Part model, mm, in its own coordinate system. Face numbers are marked on the shaded views. Round coordinates to 2 decimals unless told otherwise and drop trailing zeros. Loops run counter-clockwise (first coordinate to the right, second up) from the corner with the lowest first, then second, coordinate; pieces in that order, holes last.
from build123d import *

# Parameters (mm, degrees)
SKETCH1_W           = 176
SKETCH1_H           = 176
BOSS_EXTRUDE1_DEPTH = 30
SKETCH3_R           = 5.055
CUT_EXTRUDE1_DEPTH  = 200.047732969


with BuildPart() as part:
    # Sketch1 → Boss-Extrude1 (new body)
    with BuildSketch(Plane.XY):
        Rectangle(SKETCH1_W, SKETCH1_H)
    extrude(amount=BOSS_EXTRUDE1_DEPTH)

    # Sketch3 → Cut-Extrude1 (cut, through all)
    with BuildSketch(Plane(origin=(0, 88, 0), x_dir=(1, 0, 0), z_dir=(0, 1, 0))):
        with Locations(Location((0, -15, 0), (0, 0, 180))):
            Circle(SKETCH3_R)
    extrude(amount=-CUT_EXTRUDE1_DEPTH, mode=Mode.SUBTRACT)


solid = part.part
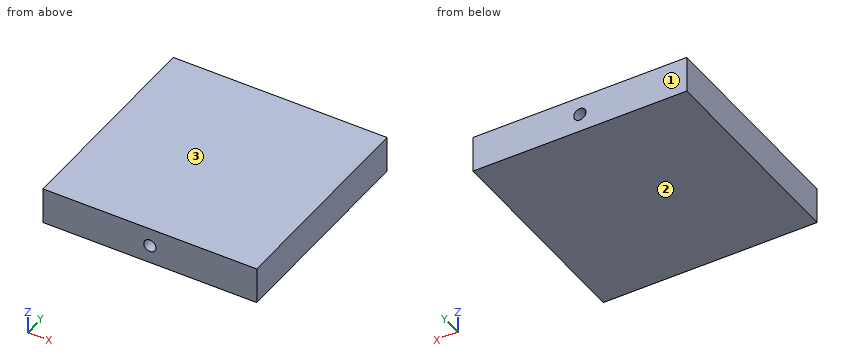
1) Mould opens along Z. For the marked faces 1, 2 and 3 say: released by +Z, released by -Z, zero draft, split by the parting line, or undercut.
Values:
face 1: zero draft
face 2: released by -Z
face 3: released by +Z
2) Slice it at B-B, the plane z = 15. Give the cut face in (x, y) (3 decimals), then the cut area to 3 significant figures.
Values:
outline: (-88, -88) - (-5.055, -88) - (-5.055, 88) - (-88, 88) - close; (5.055, -88) - (88, -88) - (88, 88) - (5.055, 88) - close
area: 29,200 mm2
3) Wall check: line 1 along Z through (x, y) = (0, -41.5) (3 decimals); line 2 along X through (y, z) = (-36.5, 14.5); line 3 along X through (y, z) = (-39, 12.5). Give the ranges that are in metal, low to high.
Values:
line 1: z = 0 to 9.945, 20.055 to 30
line 2: x = -88 to -5.03, 5.03 to 88
line 3: x = -88 to -4.39, 4.39 to 88
4) Slice it at A-A, the plane x = 0. Give the cut face in (y, z) (3 decimals), then the cut area to 3 significant figures.
Values:
outline: (-88, 0) - (88, 0) - (88, 9.945) - (-88, 9.945) - close; (-88, 20.055) - (88, 20.055) - (88, 30) - (-88, 30) - close
area: 3,500 mm2
5) Slice it at C-C, the plane y = -64. Give the cut face in (x, z) (3 decimals).
Values:
outline: (-88, 0) - (88, 0) - (88, 30) - (-88, 30) - close; hole circle Ø10.11 at (0, 15)
